```python
from build123d import *

# Parameters (mm, degrees)
SKETCH_1_W          = 120
SKETCH_1_H          = 80
EXTRUDE_1_DEPTH     = 80
SKETCH_2_R          = 5
CUT_EXTRUDE_1_DEPTH = 150.666295471
CUT_EXTRUDE_2_DEPTH = 150.666295471
CUT_EXTRUDE_3_REACH = 109.703
SKETCH_5_W          = 10
SKETCH_5_H          = 11.18
SKETCH_6_W          = 10
SKETCH_6_H          = 11.18
EXTRUDE_2_DEPTH     = 50


with BuildPart() as part:
    # 草图1 → 凸台-拉伸1 (new body)
    with BuildSketch(Plane.XY):
        Rectangle(SKETCH_1_W, SKETCH_1_H)
    extrude(amount=EXTRUDE_1_DEPTH)

    # 草图2 → 切除-拉伸1 (cut, through all)
    with BuildSketch(Plane.ZY.offset(60)):
        with Locations((40, 0)):
            Circle(SKETCH_2_R)
    extrude(amount=-CUT_EXTRUDE_1_DEPTH, mode=Mode.SUBTRACT)

    # 草图4 → 切除-拉伸2 (cut, through all)
    with BuildSketch(Plane(origin=(60, 0, 0), x_dir=(0, 0, -1), z_dir=(1, 0, 0))):
        with BuildLine():
            ThreePointArc((-80, 4.27e-07), (-75.438313853, 21.82692854), (-62.516888038, 40))
            Line((-62.516888038, 40), (-80, 40))
            Line((-80, 40), (-80, 4.27e-07))
        make_face()
        with BuildLine():
            ThreePointArc((-62.516888038, -40), (-75.438314024, -21.826928149), (-80, 4.27e-07))
            Line((-80, 4.27e-07), (-80, -40))
            Line((-80, -40), (-62.516888038, -40))
        make_face()
    extrude(amount=-CUT_EXTRUDE_2_DEPTH, mode=Mode.SUBTRACT)

    # 草图5 → 切除-拉伸3 (cut, up to next)
    with BuildSketch(Plane(origin=(0, 0, 0), x_dir=(-1, 0, 0), z_dir=(0, 0, -1)), mode=Mode.PRIVATE) as cut_extrude_3_sk1:
        Rectangle(SKETCH_5_W, SKETCH_5_H)
    cut_extrude_3_tool1 = extrude(cut_extrude_3_sk1.sketch, amount=-CUT_EXTRUDE_3_REACH, mode=Mode.PRIVATE) & part.part
    add(cut_extrude_3_tool1.solids().sort_by_distance((0, 0, 0))[0], mode=Mode.SUBTRACT)

    # 草图6 → 凸台-拉伸2 (add)
    with BuildSketch(Plane(origin=(0, 0, 0), x_dir=(-1, 0, 0), z_dir=(0, 0, -1))):
        Rectangle(SKETCH_6_W, SKETCH_6_H)
    extrude(amount=-EXTRUDE_2_DEPTH)


solid = part.part
```
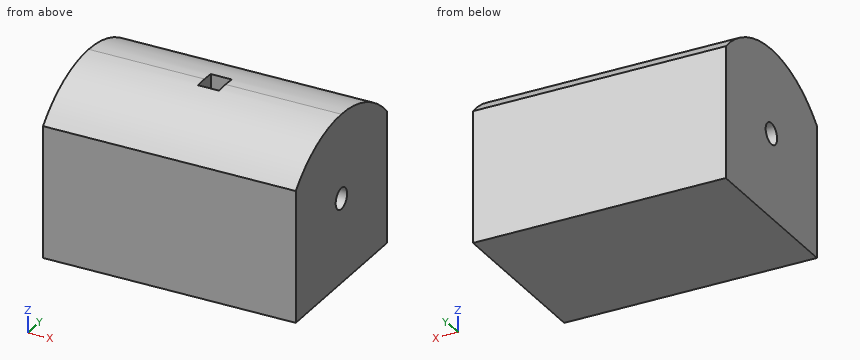
CAD build for the part. Positions are in the model's coordinates, mm. Round coordinates to 2 decimals unless told otherwise and drop trailing zeros. Write each loop counter-clockwise with the first axis right and the second up, starting at its lowest first coordinate (ties: lowest second). Pieces come first, ordered by that corner, then holes. Notation, with made-up numbers: (41, 16) - (83, 16) arc R21 cw to (83, 23) - close; hole circle Ø4 at (-15, 38.5). An arc over 180 degrees is marked (long way). Return JSON: item names as keys, results as strings. Group by question number.
Item 1: Probe probe 1 along Y at (x, z) = (22, 40); probe 2 along Y at (x, z) = (48, 35.5); probe 3 along Z at (x, y) = (12, 20). List the from-to ranges inside material, lowest first.
Item 2: Band-saw the part on B-B on x = -28. List the corners of the cut face in (y, z).
Item 3: Band-saw the part on D-D on y = 32. List the corners of the cut face in (x, z).
Item 4: Band-saw the part on A-A on z = 43. List the corners of the cut face in (x, y), plus the area to 3 significant figures.
Item 5: Flat gauge pins, fed straight in: pin 1 Ø5 at (y, z) = (-1.5, 40) entering from -X; pin 2 Ø8 at (x, y) = (-30, 10.5) entering from +Z; pin 3 Ø3 at (y, z) = (2, 38) entering from +X. Where does each tip first touch, or does it go through?
Item 6: Band-saw the part on C-C on y = -3.5. List the corners of the cut face in (x, z), plus the area to 3 significant figures.
Resolved:
{
 "1": {"probe 1": "y = -40 to -5, 5 to 40", "probe 2": "y = -40 to -2.18, 2.18 to 40", "probe 3": "z = 0 to 76.2"},
 "2": {"outline": "(-40, 0) - (40, 0) - (40, 62.52) arc R54.5 ccw to (-40, 62.52) - close; hole circle Ø10 at (0, 40)"},
 "3": {"outline": "(-60, 0) - (60, 0) - (60, 69.62) - (-60, 69.62) - close"},
 "4": {"outline": "(-60, -40) - (60, -40) - (60, -4) - (5, -4) - (5, 4) - (60, 4) - (60, 40) - (-60, 40) - (-60, 4) - (-5, 4) - (-5, -4) - (-60, -4) - close", "area": "8,720 mm²"},
 "5": {"pin 1": "stops at x = -5", "pin 2": "stops at z = 79.61", "pin 3": "stops at x = 5"},
 "6": {"outline": "(-60, 0) - (60, 0) - (60, 36.43) - (5, 36.43) - (5, 43.57) - (60, 43.57) - (60, 79.89) - (5, 79.89) - (5, 50) - (-5, 50) - (-5, 79.89) - (-60, 79.89) - (-60, 43.57) - (-5, 43.57) - (-5, 36.43) - (-60, 36.43) - close", "area": "8,500 mm²"}
}
